Answer from the drawing. Dimensions are ordinates in mm from the lowest x, y and z of the part. A direction names the side the tool comes from. Round coordinates to 2 decimals unless told otherwise and drop trailing zeros. Write each loop counter-clockwise with the first axis right and the second up, starting at its lowest first coordinate (ties: lowest second). Pieces come first, ordered by that corner, then holes. Notation, with made-up numbers: (-30.75, 60.5) -> (18.25, 60.5) arc R33 cw to (18.25, 89.5) -> close; hole circle Ø9 at (-10.5, -9). An arc over 180 degrees is marked (long way). Return JSON: item names as keys, results as strings. Group by question number.
(1) Straight lines are drawn through the part: line 1 (X direction, y = 7.5, z = 7.5); line 2 (Y direction, x = 11.25, z = 12.75); line 3 (X direction, y = 11.25, z = 9.75). For each, find the intervals that lie inside material, in ascending order.
(2) Given pin 1 (3 mm diameter, centred on x = 10, y = 3, fed in from +Z); pin 2 (1 mm diameter, centred on y = 19, z = 9.5, fed in from -X); pin 3 (6 mm diameter, centred on x = 6.5, y = 10.5, fed in from -Z), each flat-ended and moving along its own axis, determine where each tip first touches the part or whether it passes through.
(3) A cutting plane is placed at B-B on z = 7.5. Give the vertices of the cut face in (x, y), then the cut area to 3 significant figures.
(4) The mould has two halves that part along Z. Classify the marked faces 4, 5 and 6: released by +Z, released by -Z, zero draft, split by the parting line, or undercut.
(5) A cutting plane is placed at D-D on y = 16. Give the vertices of the cut face in (x, z).
(6) A cutting plane is placed at A-A on x = 7.5. Give the vertices of the cut face in (y, z), then the cut area to 3 significant figures.
(7) For the marked faces 1, 2 and 3, determine the directions among +Z, -Z, +X, -X, +Y, -Y from which every point of the face is accessible in a straight line to the end or side of a thin tool.
(8) A cutting plane is placed at C-C on y = 12.75. Give the vertices of the cut face in (x, z).
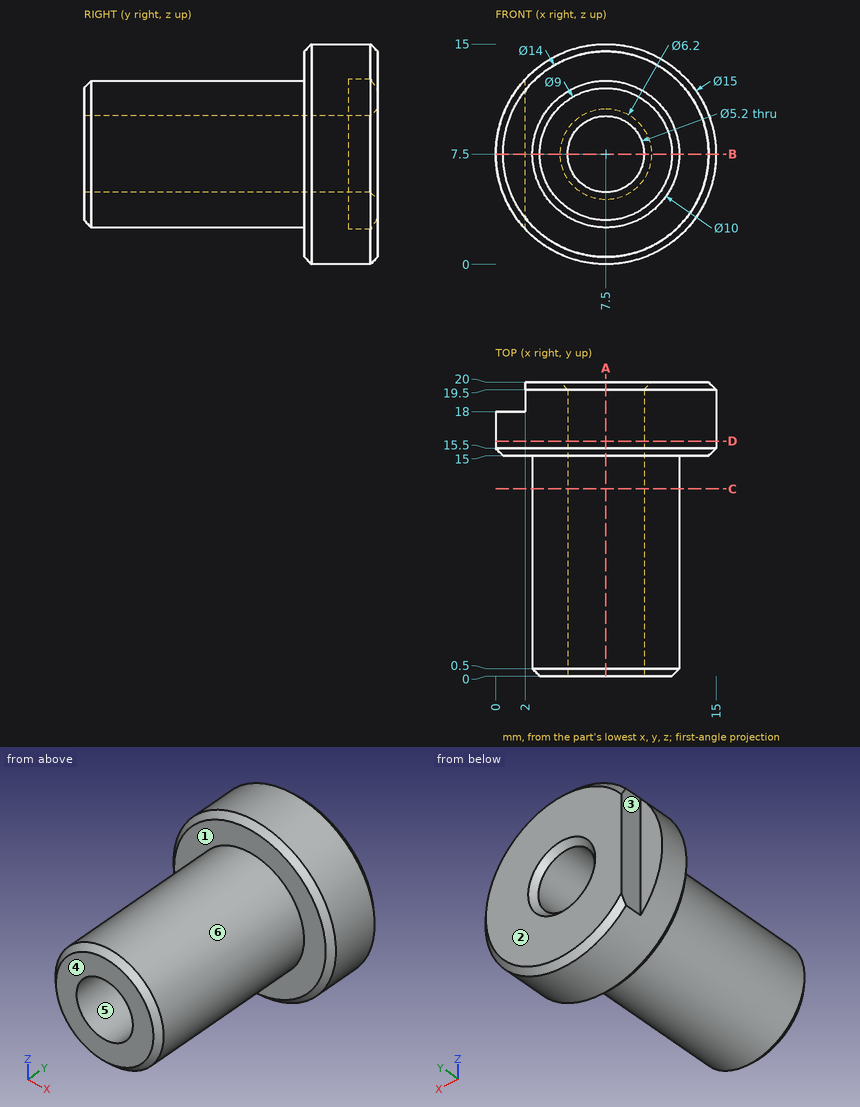
Checks:
{
 "1": {"line 1": "x = 2.5 to 4.9, 10.1 to 12.5", "line 2": "y = 15 to 20", "line 3": "x = 3.03 to 6.2, 8.8 to 11.97"},
 "2": {"pin 1": "stops at z = 12.4", "pin 2": "stops at x = 2", "pin 3": "stops at z = 2.5"},
 "3": {"outline": "(0, 15.5) -> (0.5, 15) -> (2.5, 15) -> (2.5, 0.5) -> (3, 0) -> (4.9, 0) -> (4.9, 19.5) -> (4.4, 20) -> (2, 20) -> (2, 18) -> (0, 18) -> close; (10.1, 0) -> (12, 0) -> (12.5, 0.5) -> (12.5, 15) -> (14.5, 15) -> (15, 15.5) -> (15, 19.5) -> (14.5, 20) -> (10.6, 20) -> (10.1, 19.5) -> close", "area": "116 mm^2"},
 "4": {"face 4": "zero draft", "face 5": "undercut", "face 6": "split by the parting line"},
 "5": {"outline": "circle Ø15 at (7.5, 7.5); hole circle Ø5.2 at (7.5, 7.5)"},
 "6": {"outline": "(0, 3) -> (0.5, 2.5) -> (15, 2.5) -> (15, 0.5) -> (15.5, 0) -> (19.5, 0) -> (20, 0.5) -> (20, 4.4) -> (19.5, 4.9) -> (0, 4.9) -> close; (0, 10.1) -> (19.5, 10.1) -> (20, 10.6) -> (20, 14.5) -> (19.5, 15) -> (15.5, 15) -> (15, 14.5) -> (15, 12.5) -> (0.5, 12.5) -> (0, 12) -> close", "area": "120 mm^2"},
 "7": {"face 1": "-Y", "face 2": "+Z, -Z, +X, -X, +Y", "face 3": "+Z, -Z, -X, +Y"},
 "8": {"outline": "circle Ø10 at (7.5, 7.5); hole circle Ø5.2 at (7.5, 7.5)"}
}
